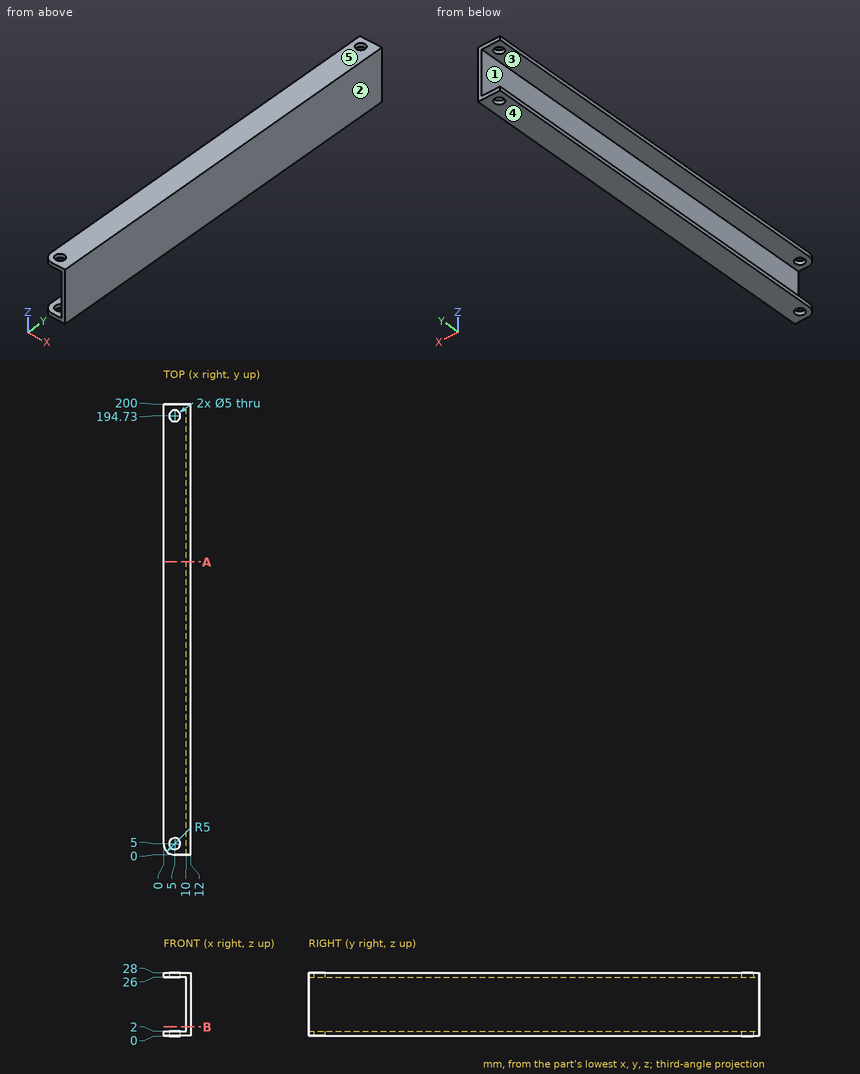
Check sheet for the drawn part. Datum: minimum x, y, z corner. Units: mm. A direction names the side the tool comes from. Round coordinates to 2 decimals unless told otherwise and drop trailing zeros. Order: outer loops, then holes, each group sorted by start corner. A loop starts at its lowest first (then second) coordinate and runs counter-clockwise, first axis right, second up. Notation, with made-up numbers: (1, 64.25) -> (10, 64.25) arc R24 ccw to (10, 103.25) -> close; hole circle Ø7 at (15, -31.75). An arc over 180 degrees is marked (long way). Put each result on its own line as item: value.
1) Depth check by flat-ended pin: pin 1 (4 mm diameter, centred on y = 73, z = 22, fed in from -X). Enter the tip coordinate at first touch or a pass-through.
Final values:
pin 1: stops at x = 10
2) Mould release check, pull along Z, two halves, no side actions. Record for the marked faces 3, 4 and 5: +Z half, -Z half, draft (parallel to the pull), parting line (faces both ways), or undercut.
Final values:
face 3: undercut
face 4: -Z half
face 5: +Z half
3) Section check B-B (z = 4). Record the cut outline in (x, y), then the cut area to 3 significant figures.
Final values:
outline: (10, 0) -> (12, 0) -> (12, 200) -> (10, 200) -> close
area: 400 mm^2
4) Section check A-A (y = 130). Record the cut outline in (x, z).
Final values:
outline: (0, 0) -> (12, 0) -> (12, 28) -> (0, 28) -> (0, 26) -> (10, 26) -> (10, 2) -> (0, 2) -> close
5) Material ranges on line 1 (Y direction, x = 5, z = 27.2); line 2 (Z direction, x = 1.5, y = 51.5); line 3 (X direction, y = 5, z = 26.4), recorded low to high.
Final values:
line 1: y = 0 to 2.5, 7.5 to 192.23, 197.23 to 200
line 2: z = 0 to 2, 26 to 28
line 3: x = 0 to 2.5, 7.5 to 12
6) Set-up check for the marked faces 1 and 2: record each of +Z, -Z, +X, -X, +Y, -Y from which the full face is reachable in a straight line by a thin tool's end or side.
Final values:
face 1: -X, +Y, -Y
face 2: +Z, -Z, +X, +Y, -Y
